For this review, use the dimensioned drawing (mm, ordinates from the lowest corner) and the shaded views. A direction names the side the tool comes from. Round coordinates to 2 decimals unless told otherwise and drop trailing zeros. Write each loop counter-clockwise with the first axis right and the second up, starting at its lowest first coordinate (ties: lowest second). Pieces come first, ordered by that corner, then holes.
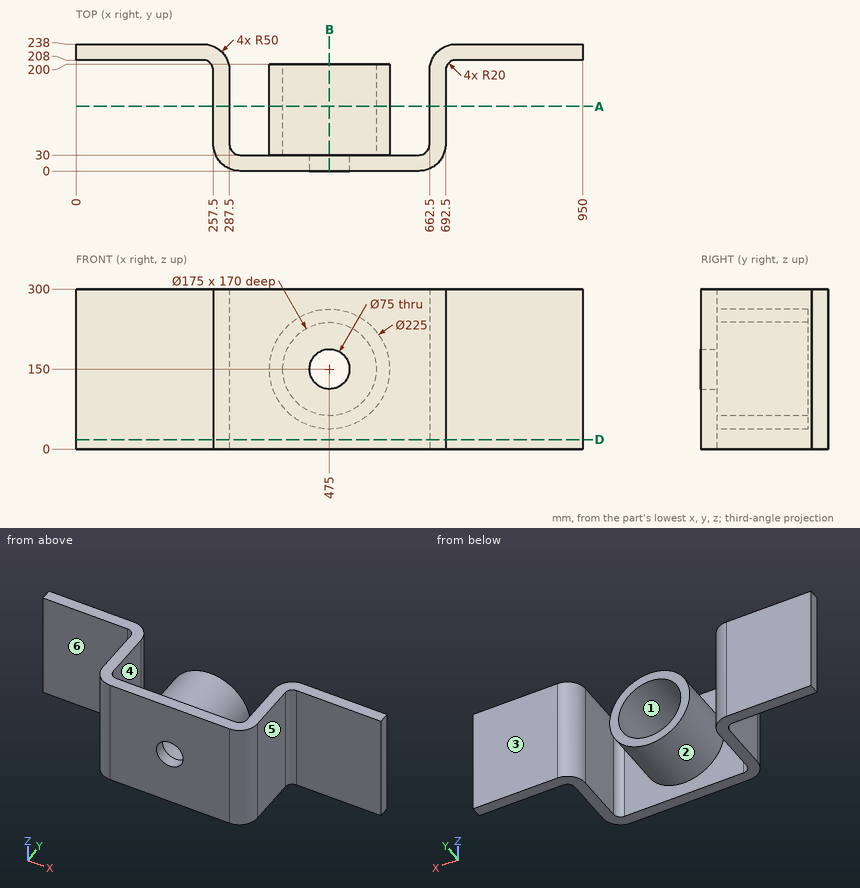
1) For P1, Ø5, axis at x = 369.5, y = 124, coming from the -Z side; P2, Ø2, axis at x = 826.5, z = 67, coming from the -Y side; P3, Ø12, axis at x = 563, z = 135.5, coming from the +Y side, all flat-tipped, find the tip position at first contact; note any pin that passes through.
2) Add section B-B on x = 475. State the section outline as (y, z) points, and give its area (4 significant figures).
3) For line 1 along Z through (x, y) = (475, 20.75); line 2 along X through (y, z) = (42, 48); line 3 along X through (y, z) = (168, 61.5), list the stretches that pass through material, from the lowest coordinate up.
4) Add section D-D on z = 18. State the section outline as (x, y) points, and give its area (3 significant figures).
5) Add section A-A on y = 121. State the section outline as (x, z) points.
6) The part is to be moulded in two halves that separate along Z. For the marked faces 1, 2 and 3, say which applies: pulls with the +Z half, pulls with the -Z half, needs draft (parallel to the pull), parting line crosses it, or undercut.
7) For the marked faces 4, 5 and 6, list the 3-axis set-ups (+Z, -Z, +X, -X, +Y, -Y) from which the entire face can be reached by the end or side of a thin tool; tool diameter is ignored.
Computed:
1. P1: stops at z = 104.75
1. P2: stops at y = 208
1. P3: stops at y = 200
2. outline: (0, 0) - (30, 0) - (30, 37.5) - (200, 37.5) - (200, 62.5) - (30, 62.5) - (30, 112.5) - (0, 112.5) - close; (0, 187.5) - (30, 187.5) - (30, 237.5) - (200, 237.5) - (200, 262.5) - (30, 262.5) - (30, 300) - (0, 300) - close
2. area: 15,250 mm2
3. line 1: z = 0 to 112.5, 187.5 to 300
3. line 2: x = 258.14 to 289.17, 427.54 to 522.46, 660.83 to 691.86
3. line 3: x = 257.5 to 287.5, 405.54 to 544.46, 662.5 to 692.5
4. outline: (0, 208) - (237.5, 208) arc R20 cw to (257.5, 188) - (257.5, 50) arc R50 ccw to (307.5, 0) - (642.5, 0) arc R50 ccw to (692.5, 50) - (692.5, 188) arc R20 cw to (712.5, 208) - (950, 208) - (950, 238) - (712.5, 238) arc R50 ccw to (662.5, 188) - (662.5, 50) arc R20 cw to (642.5, 30) - (307.5, 30) arc R20 cw to (287.5, 50) - (287.5, 188) arc R50 ccw to (237.5, 238) - (0, 238) - close
4. area: 39,200 mm2
5. outline: (257.5, 0) - (287.5, 0) - (287.5, 300) - (257.5, 300) - close; circle Ø225 at (475, 150); (662.5, 0) - (692.5, 0) - (692.5, 300) - (662.5, 300) - close; hole circle Ø175 at (475, 150)
6. face 1: undercut
6. face 2: parting line crosses it
6. face 3: needs draft
7. face 4: +Z, -Z, +Y
7. face 5: +Z, -Z, +X, -Y
7. face 6: +Z, -Z, -X, -Y
